```python
from build123d import *

# Parameters (mm, degrees)
SKETCH1_R           = 8
BOSS_EXTRUDE1_DEPTH = 198.5
SKETCH2_R           = 6
BOSS_EXTRUDE2_DEPTH = 30
BOSS_EXTRUDE3_START = 60
SKETCH3_R           = 6
BOSS_EXTRUDE3_DEPTH = 60
CHAMFER1_SIZE       = 1
CHAMFER2_SIZE       = 1


with BuildPart() as part:
    # Sketch1 → Boss-Extrude1 (new, symmetric)
    with BuildSketch(Plane(origin=(0, 0, 0), x_dir=(0, 0, -1), z_dir=(1, 0, 0))):
        Circle(SKETCH1_R)
    extrude(amount=BOSS_EXTRUDE1_DEPTH, both=True)

    # Sketch2 → Boss-Extrude2 (add)
    with BuildSketch(Plane(origin=(198.5, 0, 0), x_dir=(0, 0, -1), z_dir=(1, 0, 0))):
        Circle(SKETCH2_R)
    extrude(amount=BOSS_EXTRUDE2_DEPTH)

    # Sketch3 → Boss-Extrude3 (add)
    with BuildSketch(Plane.ZY.offset(198.5).offset(BOSS_EXTRUDE3_START)):
        with Locations(Location((0, 0, 0), (0, 0, 180))):
            Circle(SKETCH3_R)
    extrude(amount=-BOSS_EXTRUDE3_DEPTH)

    # Chamfer1
    chamfer1_edges = [part.edges().sort_by_distance(p)[0] for p in [
        (228.5, 0, 6),
    ]]
    chamfer(chamfer1_edges, length=CHAMFER1_SIZE)

    # Chamfer2
    chamfer2_edges = [part.edges().sort_by_distance(p)[0] for p in [
        (-258.5, 0, 6),
    ]]
    chamfer(chamfer2_edges, length=CHAMFER2_SIZE)


solid = part.part
```
Can you work these out from the model? Positions are in its coordinate system, mm. A direction names the side the tool comes from. Round coordinates to 2 decimals unless told otherwise and drop trailing zeros. Loops run counter-clockwise (first coordinate to the right, second up) from the corner with the lowest first, then second, coordinate; pieces in that order, holes last. Notation, with made-up numbers: (39.25, 72) -> (95.25, 72) arc R32 ccw to (95.25, 102) -> close; hole circle Ø5 at (-21, 59). An arc over 180 degrees is marked (long way). Answer in a Markdown table with one row per item.
Item 1: If I drill on probe 1 along Z at (x, y) = (-17, 1); probe 2 along X at (y, z) = (1.25, -6); probe 3 along Z at (x, y) = (111, 0.5), over which ranges is the centre line in solid material (lowest first)?
Answer block:
| item | result |
|---|---|
| probe 1 | -7.94 to 7.94 |
| probe 2 | -198.5 to 198.5 |
| probe 3 | -7.98 to 7.98 |
Item 2: Suppose I cut it at B-B, the plane x = 105.5. List the corners of the cut face in (y, z) for me.
Answer block:
| item | result |
|---|---|
| outline | circle Ø16 at (0, 0) |
Item 3: Will these pins go through, and if not, where does the flat tip stop? P1, Ø2, axis at y = 3, z = 6, coming from the +X side; P2, Ø1.5, axis at y = 6, z = 3, coming from the -X side; P3, Ø1.5, axis at x = 135, y = -3, coming from the -Z side.
Answer block:
| item | result |
|---|---|
| P1 | x = 227.79 |
| P2 | x = -257.54 |
| P3 | z = -7.68 |
Item 4: Suppose I cut it at A-A, the plane z = 0. List the corners of the cut face in (x, y) for me, plus the area to 3 significant figures.
Answer block:
| item | result |
|---|---|
| outline | (-258.5, -5) -> (-257.5, -6) -> (-198.5, -6) -> (-198.5, -8) -> (198.5, -8) -> (198.5, -6) -> (227.5, -6) -> (228.5, -5) -> (228.5, 5) -> (227.5, 6) -> (198.5, 6) -> (198.5, 8) -> (-198.5, 8) -> (-198.5, 6) -> (-257.5, 6) -> (-258.5, 5) -> close |
| area | 7,430 mm² |
Item 5: On a 3-axis mill with a long thin cutter (end or side, diameter ignored), from which of +Z, -Z, +X, -X, +Y, -Y can I reach the whole of each face in a straight line? I mean faces 1 (the cylindrical face through (2.78, -7.81, 1.73)), 2 (the cylindrical face through (213, 0, 6)), 3 (the flat face through (-198.5, 6, 2)). Say none if no direction works.
Answer block:
| item | result |
|---|---|
| face 1 | +X, -X |
| face 2 | +X |
| face 3 | -X |
